from build123d import *

# Parameters (mm, degrees)
SKETCH1_R             = 480
SKETCH1_R_2           = 375
BOSS_EXTRUDE1_DEPTH   = 6
CUT_EXTRUDE3_REACH    = 680.849
SKETCH2_W             = 12
SKETCH2_H             = 500
CIRPATTERN1_COUNT     = 3
M8_TAPPED_HOLE1_D     = 6.8
M8_TAPPED_HOLE1_DEPTH = 6


with BuildPart() as part:
    # Sketch1 → Boss-Extrude1 (new body)
    with BuildSketch(Plane(origin=(0, 0, 0), x_dir=(1, 0, 0), z_dir=(0, 1, 0))):
        with Locations(Location((0, 0, 0), (0, 0, 270))):
            Circle(SKETCH1_R)
        with Locations(Location((0, 0, 0), (0, 0, 270))):
            Circle(SKETCH1_R_2, mode=Mode.SUBTRACT)
    extrude(amount=BOSS_EXTRUDE1_DEPTH)

    # Sketch2 → Cut-Extrude3 (cut, up to next)
    with BuildSketch(Plane(origin=(0, 0, 0), x_dir=(1, 0, 0), z_dir=(0, 1, 0)), mode=Mode.PRIVATE) as cut_extrude3_sk1:
        with Locations((-480, 0)):
            Rectangle(SKETCH2_W, SKETCH2_H)
    cut_extrude3_tool1 = extrude(cut_extrude3_sk1.sketch, amount=CUT_EXTRUDE3_REACH, mode=Mode.PRIVATE) & part.part
    # Sketch2 → Cut-Extrude3 (cut, up to next)
    with BuildSketch(Plane(origin=(0, 0, 0), x_dir=(1, 0, 0), z_dir=(0, 1, 0)), mode=Mode.PRIVATE) as cut_extrude3_sk2:
        with Locations((480, 0)):
            Rectangle(SKETCH2_W, SKETCH2_H)
    cut_extrude3_tool2 = extrude(cut_extrude3_sk2.sketch, amount=CUT_EXTRUDE3_REACH, mode=Mode.PRIVATE) & part.part
    cut_extrude3_1 = cut_extrude3_tool1.solids().sort_by_distance((-480, 0, 0))[0]
    add(cut_extrude3_1, mode=Mode.SUBTRACT)
    cut_extrude3_2 = cut_extrude3_tool2.solids().sort_by_distance((480, 0, 0))[0]
    add(cut_extrude3_2, mode=Mode.SUBTRACT)
    cut_extrude3 = cut_extrude3_1 + cut_extrude3_2  # Cut-Extrude3 as one shape, for the pattern or mirror that repeats it

    # CirPattern1: Cut-Extrude3 ×3 about axis
    cirpattern1_axis = Axis((0, 0, 0), (0, 1, 0))
    for i in range(1, CIRPATTERN1_COUNT):
        add(cut_extrude3.rotate(cirpattern1_axis, i * 360 / CIRPATTERN1_COUNT), mode=Mode.SUBTRACT)

    # M8 Tapped Hole1
    with Locations(Plane(origin=(0, 6, 0), x_dir=(1, 0, 0), z_dir=(0, 1, 0))):
        with Locations((0, 430), (111.292189394, 415.348105304), (-111.292189394, 415.348105304), (372.390923627, 215), (415.348105304, 111.292189394), (304.05591591, 304.05591591), (372.390923627, -215), (304.05591591, -304.05591591), (415.348105304, -111.292189394), (0, -430), (-111.292189394, -415.348105304), (111.292189394, -415.348105304), (-372.390923627, -215), (-415.348105304, -111.292189394), (-304.05591591, -304.05591591), (-372.390923627, 215), (-304.05591591, 304.05591591), (-415.348105304, 111.292189394), (0, 0)):
            Hole(M8_TAPPED_HOLE1_D / 2, depth=M8_TAPPED_HOLE1_DEPTH)


solid = part.part
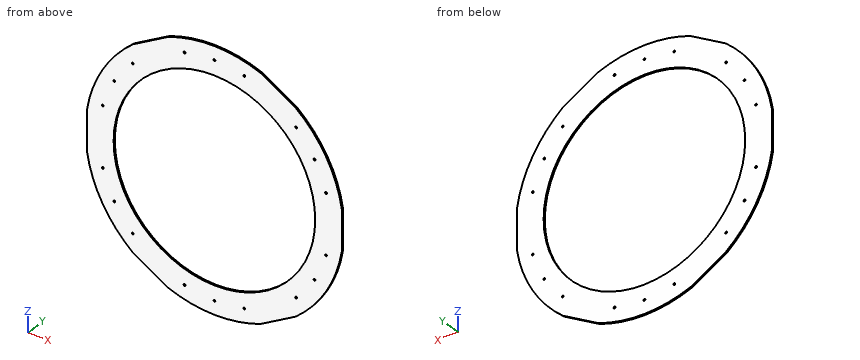
Source: CAD feature listing. Evaluate the final solid. Frame: model axes, mm. Round coordinates to 2 decimals unless told otherwise and drop trailing zeros. Loops run counter-clockwise (first coordinate to the right, second up) from the corner with the lowest first, then second, coordinate; pieces in that order, holes last. Notation, with made-up numbers: (61, 23.5) - (88, 23.5) arc R31 ccw to (88, 54.5) - close; hole circle Ø8 at (61, 63). An arc over 180 degrees is marked (long way). Write item = value, one per line. Start each with the question number.
(1) Pin query (flat end, axial travel): pin 1 (1.5 mm diameter, centred on x = -372.5, y = 3.5, fed in from -Z); pin 2 (11 mm diameter, centred on x = 304.06, z = -304.06, fed in from +Y); pin 3 (3 mm diameter, centred on x = 79.5, y = 1.5, fed in from +Z); pin 4 (3 mm diameter, centred on y = 2.5, z = 97, fed in from +X). Return the tip coordinate at first contact, or that it passes through.
(2) Section query B-B, the plane x = -338.5. Output: boundary loops of the cut face in (y, z).
(3) Ray query, line 1 along X through (y, z) = (4, 215); line 2 along Z through (x, y) = (305.5, 3); line 3 along Z through (x, y) = (41, 3.45). Return the intervals inside material, ascending. Write a range as from..to.
(4) Section query A-A, the plane z = 0. Output: boundary loops of the cut face in (x, y), plus the area to 3 significant figures.
(5) Section query C-C, the plane y = 2.55. State how many separate pieces and enclosed holes the cut face has, plus the area to 3 significant figures.
Conclusion:
q1.pin_1 = -303.65
q1.pin_2 = 6
q1.pin_3 = 473.62
q1.pin_4 = 470.4
q2.outline = (0, -340.32) - (6, -340.32) - (6, -161.38) - (0, -161.38) - close; (0, 161.38) - (6, 161.38) - (6, 340.32) - (0, 340.32) - close
q3.line_1 = -429.16..-375.79, -368.99..-307.25, 307.25..368.99, 375.79..429.16
q3.line_2 = -370.23..-307.13, -300.98..-217.47, 217.47..300.98, 307.13..370.23
q3.line_3 = -478.25..-372.75, 372.75..478.25
q4.outline = (-474, 0) - (-375, 0) - (-375, 6) - (-474, 6) - close; (375, 0) - (474, 0) - (474, 6) - (375, 6) - close
q4.area = 1,190 mm2
q5.separate_pieces = 1
q5.enclosed_holes = 19
q5.area = 278,000 mm2
